Design review of the part built by this model. Coordinates are the model's own, in mm. A direction names the side the tool comes from. Give positions to 0.01 mm unless a question says otherwise; leave off trailing zeros. Order: outer loops, then holes, each group sorted by start corner. A loop starts at its lowest first (then second) coordinate and runs counter-clockwise, first axis right, second up. Notation, with made-up numbers: (1.5, 36) -> (55.5, 36) arc R25 ccw to (55.5, 49) -> close; hole circle Ø6 at (36, -26.75). An arc over 180 degrees is marked (long way). Answer in a Markdown table with one row per item. Add a question column.
```python
from build123d import *

# Parameters (mm, degrees)
SKETCH_1_W                = 100
SKETCH_1_H                = 35
EXTRUDE_1_DEPTH           = 12
CHAMFER_1_SIZE            = 15
CHAMFER_1_SIZE2           = 8.660254038
HOLE_WIZARD_1_D           = 5.5
HOLE_WIZARD_1_CBORE_D     = 10
HOLE_WIZARD_1_CBORE_DEPTH = 5.7


with BuildPart() as part:
    # 草图1 → 凸台-拉伸1 (new body)
    with BuildSketch(Plane.XY):
        Rectangle(SKETCH_1_W, SKETCH_1_H)
    extrude(amount=EXTRUDE_1_DEPTH)

    # 倒角1
    chamfer_1_edges = [part.edges().sort_by_distance(p)[0] for p in [
        (50, -17.5, 6),
        (-50, -17.5, 6),
    ]]
    chamfer_1_side = [part.faces().sort_by_distance(p)[0] for p in [
        (0, -17.5, 6),
    ]]
    chamfer(chamfer_1_edges, length=CHAMFER_1_SIZE, length2=CHAMFER_1_SIZE2, reference=chamfer_1_side[0])

    # 打孔尺寸(%根据)内六角圆柱头螺钉的类型1 (through all)
    with Locations(Plane(origin=(0, 0, 0), x_dir=(-1, 0, 0), z_dir=(0, 0, -1))):
        with Locations((0, 10.5), (0, -7.5)):
            CounterBoreHole(HOLE_WIZARD_1_D / 2, HOLE_WIZARD_1_CBORE_D / 2, HOLE_WIZARD_1_CBORE_DEPTH)


solid = part.part
```
1) Machinability: for faces 4 (the face through (-50, 4, 6)), 5 (the face through (0.651, -2.543, 2.81)), which of the approach directions +Z, -Z, +X, -X, +Y, -Y give a long, thin tool a straight path to every point of the face, cutting with its end or side? Answer none if there is none.
2) Mouldability with a two-part tool opening along X and no side actions: class faces 1 (the face through (-0.596, -10.185, 8.894)), 2 (the face through (50, 4, 6)), 3 (the face through (-1, 0, 0)) as +X half, -X half, draft (parallel to the pull), parting line (faces both ways), or undercut.
3) For L1, parallel to Y at x = 0, z = 4.6; L2, parallel to Y at x = 0, z = 8.25; L3, parallel to X at y = 9, z = 2.25, list the stretches that pass through material, from the lowest coordinate up.
4) Add section C-C, the plane y = 10.5. Write out the cut boundary in (x, z), and give its area (3 significant figures).
5) Add section B-B, the plane z = 11. Write out the cut boundary in (x, y).
6) Clearance check with flat-ended pins moving along their axes: P1, Ø3, axis at x = 2, y = 10, coming from the -Z side; P2, Ø4.5, axis at x = 0, y = 10.5, coming from the +Z side. State where each tip first meets the part, or that it passes through.
7) Add section A-A, the plane x = 0. Write out the cut boundary in (y, z).
8) Add section D-D, the plane z = 4.25. Write out the cut boundary in (x, y), and give its area (3 significant figures).
Verdict:
| question | item | result |
|---|---|---|
| 1 | face 4 | +Z, -Z, -X, +Y, -Y |
| 1 | face 5 | -Z |
| 2 | face 1 | undercut |
| 2 | face 2 | +X half |
| 2 | face 3 | draft |
| 3 | L1 | y = -17.5 to -12.5, -2.5 to 5.5, 15.5 to 17.5 |
| 3 | L2 | y = -17.5 to -10.25, -4.75 to 7.75, 13.25 to 17.5 |
| 3 | L3 | x = -50 to -4.77, 4.77 to 50 |
| 4 | outline | (-50, 0) -> (-5, 0) -> (-5, 5.7) -> (-2.75, 5.7) -> (-2.75, 12) -> (-50, 12) -> close; (2.75, 5.7) -> (5, 5.7) -> (5, 0) -> (50, 0) -> (50, 12) -> (2.75, 12) -> close |
| 4 | area | 1,110 mm2 |
| 5 | outline | (-50, -8.84) -> (-35, -17.5) -> (35, -17.5) -> (50, -8.84) -> (50, 17.5) -> (-50, 17.5) -> close; hole circle Ø5.5 at (0, -7.5); hole circle Ø5.5 at (0, 10.5) |
| 6 | P1 | stops at z = 5.7 |
| 6 | P2 | passes through |
| 7 | outline | (-17.5, 0) -> (-12.5, 0) -> (-12.5, 5.7) -> (-10.25, 5.7) -> (-10.25, 12) -> (-17.5, 12) -> close; (-4.75, 5.7) -> (-2.5, 5.7) -> (-2.5, 0) -> (5.5, 0) -> (5.5, 5.7) -> (7.75, 5.7) -> (7.75, 12) -> (-4.75, 12) -> close; (13.25, 5.7) -> (15.5, 5.7) -> (15.5, 0) -> (17.5, 0) -> (17.5, 12) -> (13.25, 12) -> close |
| 8 | outline | (-50, -8.84) -> (-35, -17.5) -> (35, -17.5) -> (50, -8.84) -> (50, 17.5) -> (-50, 17.5) -> close; hole circle Ø10 at (0, -7.5); hole circle Ø10 at (0, 10.5) |
| 8 | area | 3,210 mm2 |
